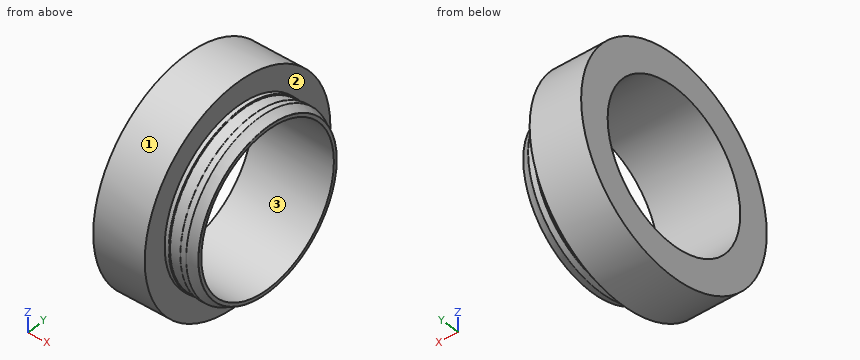
```python
from build123d import *


with BuildPart() as part:
    # Sketch2 → Revolve1 (revolve)
    with BuildSketch(Plane.XY):
        with BuildLine():
            Line((169.439894657, 49.5), (166.196302637, 49.5))
            ThreePointArc((166.196302637, 49.5), (166.054881281, 49.441421356), (165.996302637, 49.3))
            Line((165.996302637, 49.3), (165.996302637, 49.2))
            ThreePointArc((165.996302637, 49.2), (165.937723993, 49.058578644), (165.796302637, 49))
            Line((165.796302637, 49), (159.696302637, 49))
            ThreePointArc((159.696302637, 49), (159.554881281, 49.058578644), (159.496302637, 49.2))
            Line((159.496302637, 49.2), (159.496302637, 49.3))
            ThreePointArc((159.496302637, 49.3), (159.437723993, 49.441421356), (159.296302637, 49.5))
            Line((159.296302637, 49.5), (156.996302637, 49.5))
            Line((156.996302637, 49.5), (156.996302637, 63))
            Line((156.996302637, 63), (126.996302637, 63))
            Line((126.996302637, 63), (126.996302637, 45))
            Line((126.996302637, 45), (174.496302637, 45))
            Line((174.496302637, 45), (174.496302637, 46.864333756))
            ThreePointArc((174.496302637, 46.864333756), (174.461934034, 46.976432999), (174.370640233, 47.050005299))
            ThreePointArc((174.370640233, 47.050005299), (171.90655177, 48.158837504), (169.544248857, 49.470617118))
            ThreePointArc((169.544248857, 49.470617118), (169.494100636, 49.492514186), (169.439894657, 49.5))
        make_face()
    revolve(axis=Axis((362.346302637, 0, 0), (-1, 0, 0)))


solid = part.part
```
Geometry: final body of the model. Coordinates: model frame, mm. Face numbers are marked on the shaded views. Round coordinates to 2 decimals unless told otherwise and drop trailing zeros. Order: outer loops, then holes, each group sorted by start corner. A loop starts at its lowest first (then second) coordinate and runs counter-clockwise, first axis right, second up. Notation, with made-up numbers: (25.25, 20) - (44.25, 20) arc R26 ccw to (44.25, 38) - close; hole circle Ø9 at (14, 39). An arc over 180 degrees is marked (long way). Write item = value, one per line. Start each with the question number.
Q1. Cut plane D-D on z = 51.5. Return the cut outline in (x, y), and give its area (3 significant figures).
Q2. Cut plane C-C on x = 146. Return the cut outline in (y, z), and give its area (3 significant figures).
Q3. Pull-direction query (Z, two-part tool) for the marked faces 1, 2 and 3; classes: +Z half, -Z half, draft (parallel to the pull), parting line (faces both ways), or undercut.
Q4. Ray query, line 1 (Y direction, x = 144, z = 0); line 2 (Y direction, x = 164, z = 0). Return the intervals inside material, ascending. Write a range as from..to.
Q5. Pin query (flat end, axial travel): pin 1 (2 mm diameter, centred on x = 160, y = 26, fed in from +Z); pin 2 (10 mm diameter, centred on x = 139.5, y = -39, fed in from -Z); pin 3 (1.5 mm diameter, centred on x = 158, y = -12, fed in from +Z). Return the tip coordinate at first contact, or that it passes through.
Outcome:
q1.outline = (127, -36.29) - (157, -36.29) - (157, 36.29) - (127, 36.29) - close
q1.area = 2,180 mm^2
q2.outline = circle Ø126 at (0, 0); hole circle Ø90 at (0, 0)
q2.area = 6,110 mm^2
q3.face_1 = parting line
q3.face_2 = draft
q3.face_3 = undercut
q4.line_1 = -63..-45, 45..63
q4.line_2 = -49..-45, 45..49
q5.pin_1 = 42.58
q5.pin_2 = -53.04
q5.pin_3 = 48.2
